The drawing under review shows one solid part. Ordinate dimensions are in mm from its lowest x, y, z. Coordinates: 2 decimals unless noted, no trailing zeros. Order: outer loops, then holes, each group sorted by start corner. A loop starts at its lowest first (then second) coordinate and runs counter-clockwise, first axis right, second up. Notation, with made-up numbers: M 56.25,12 L 72.25,12 A21 cw 72.25,42 Z; hole C -32.75,-30.5 d4. An arc over 180 degrees is marked long. Answer as a JSON object with one key per item and string values.
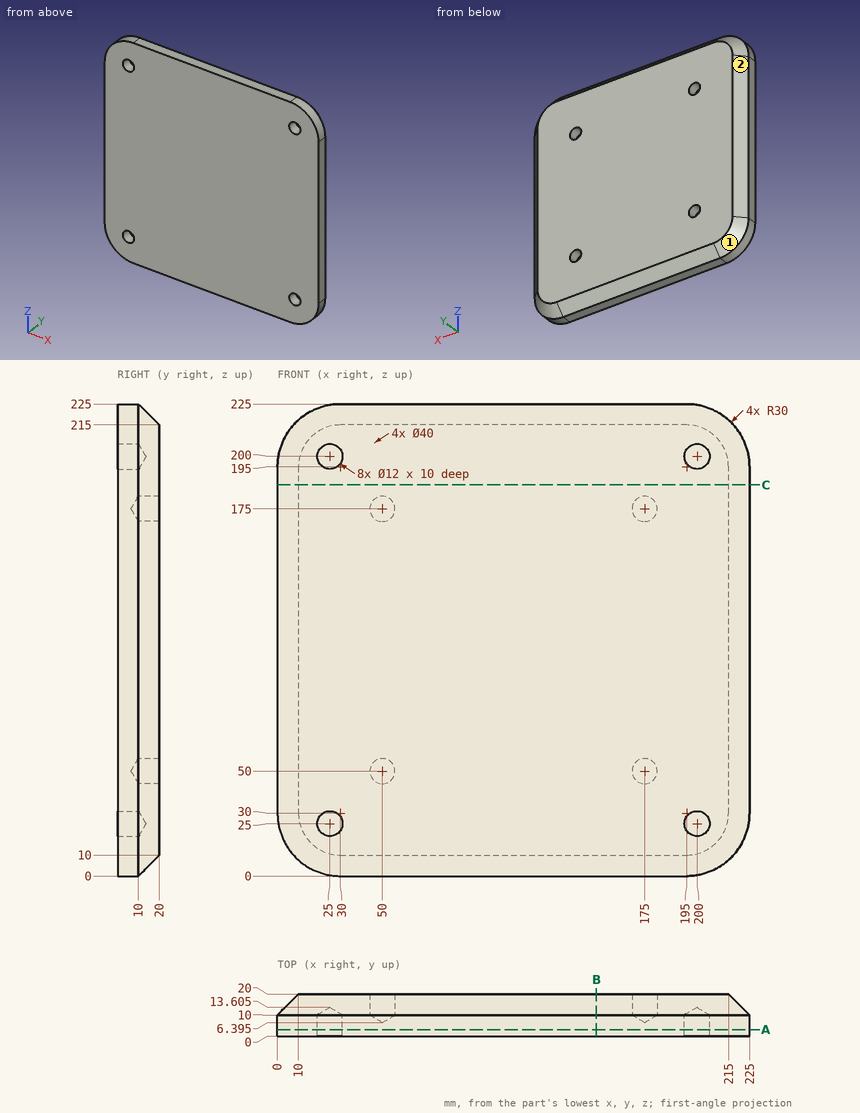
1) Add section A-A (y = 3). State the section outline as (x, z) points, and give its area (3 significant figures).
Taken from the geometry:
{"outline": "M 0,30 A30 ccw 30,0 L 195,0 A30 ccw 225,30 L 225,195 A30 ccw 195,225 L 30,225 A30 ccw 0,195 Z; hole C 25,25 d12; hole C 25,200 d12; hole C 200,25 d12; hole C 200,200 d12", "area": "49,400 mm2"}
2) To check wall thickness, follow L1, parallel to Z at x = 25, y = 7.5; L2, parallel to X at y = 5.5, z = 26.5 (1 decimal); L3, parallel to Z at x = 50, y = 18. State the ranges of each line that lie inside material, in increasing order.
Taken from the geometry:
{"L1": "z = 0.42 to 19, 31 to 194, 206 to 224.58", "L2": "x = 0.2 to 19.2, 30.8 to 194.2, 205.8 to 224.8", "L3": "z = 8 to 44, 56 to 169, 181 to 217"}
3) Mouldability with a two-part tool opening along Z and no side actions: class the marked faces 1 and 2 as released by +Z, released by -Z, zero draft, split by the parting line, or undercut.
Taken from the geometry:
{"face 1": "released by -Z", "face 2": "zero draft"}
4) Add section C-C (z = 186.5). State the section outline as (x, y) points, and give its area (3 significant figures).
Taken from the geometry:
{"outline": "M 0,0 L 225,0 L 225,10 L 215,20 L 10,20 L 0,10 Z", "area": "4,400 mm2"}
5) Insertion check: pin 1 Ø9.5 at (x, z) = (200, 200) entering from -Y; pin 2 Ø1 at (x, z) = (201.5, 98) entering from -Y; pin 3 Ø11 at (x, z) = (200, 25) entering from -Y; pin 4 Ø8 at (y, z) = (15.5, 189.5) entering from +X. Each pin has a flat end and moves straight along its axis. Give the tip position at first contact, or say it passes through.
Taken from the geometry:
{"pin 1": "stops at y = 10.75", "pin 2": "stops at y = 0", "pin 3": "stops at y = 10.3", "pin 4": "stops at x = 223.5"}
6) Add section B-B (x = 152). State the section outline as (y, z) points.
Taken from the geometry:
{"outline": "M 0,0 L 10,0 L 20,10 L 20,215 L 10,225 L 0,225 Z"}
